Design review of the part built by this model. Coordinates are the model's own, in mm. A direction names the side the tool comes from. Give positions to 0.01 mm unless a question says otherwise; leave off trailing zeros. Loops run counter-clockwise (first coordinate to the right, second up) from the corner with the lowest first, then second, coordinate; pieces in that order, holes last. Notation, with made-up numbers: M 47.25,61 L 80.25,61 A19 ccw 80.25,81 Z; hole C -37.75,51.25 d3. An arc over 180 degrees is marked long. Use a Markdown table: item, result. Add a question column.
(1) Add section A-A, the plane x = -315. Give the boundary of the cut face in (y, z), then the cut area to 3 significant figures.
(2) Add section C-C, the plane y = -566. Give the boundary of the cut face in (x, z).
(3) Draft analysis for pull direction Y (two halves, no side actions). For faces 4 (the face through (0, -309, -7)), 5 (the face through (-358, 0, 38)), 6 (the face through (-355, -1, 75)), state which applies: pulls with the +Y half, pulls with the -Y half, needs draft (parallel to the pull), parting line crosses it, or undercut.
(4) Add section B-B, the plane x = -155. Give the boundary of the cut face in (y, z).
(5) Add section D-D, the plane y = -408.5. Give the boundary of the cut face in (x, z).
(6) For faces 1 (the face through (-348.058, -140.941, -14.953)), 2 (the face through (-707.014, -305.559, 5.517)), 3 (the face through (-358, -618, -33)), list the 3-axis set-ups (+Z, -Z, +X, -X, +Y, -Y) from which the entire face can be reached by the end or side of a thin tool; tool diameter is ignored.
(7) For probe 1 along X at (y, z) = (-585.5, -31); probe 2 along Y at (x, z) = (-285.5, 33.5); probe 3 along Z at (x, y) = (-283, -518), list the stretches that pass through material, from the lowest coordinate up.
(8) Insertion check: pin 1 Ø3 at (x, z) = (-502.5, 2.5) entering from +Y; pin 2 Ø1 at (x, y) = (1, -610.5) entering from +Z; pin 3 Ø10 at (x, y) = (-428.5, -477.5) entering from -Z. Each pin has a flat end and moves straight along its axis. Give the tip position at first contact, or say it passes through.
```python
from build123d import *

# Parameters (mm, degrees)
BOSS_EXTRUDE1_DEPTH = 2
BOSS_EXTRUDE2_DEPTH = 706
SKETCH3_W           = 706
SKETCH3_H           = 73
CUT_EXTRUDE1_DEPTH  = 940.955850027
BOSS_EXTRUDE3_START = 2
BOSS_EXTRUDE3_DEPTH = 2
CUT_EXTRUDE2_REACH  = 951.714
SKETCH5_W           = 628
SKETCH5_H           = 323
SKETCH6_W           = 100
SKETCH6_H           = 80
SKETCH6_W_2         = 344
CUT_EXTRUDE3_DEPTH  = 2
SKETCH7_W           = 706
SKETCH7_H           = 4
BOSS_EXTRUDE4_DEPTH = 61


with BuildPart() as part:
    # Sketch1 → Boss-Extrude1 (new body)
    with BuildSketch(Plane(origin=(0, 0, 0), x_dir=(0, 0, -1), z_dir=(1, 0, 0))):
        with BuildLine():
            Line((0, 0), (-75, 0))
            Line((-75, 0), (-75, -40))
            ThreePointArc((-75, -40), (-39.844354311, -53.471133381), (-31.447716035, -90.171096924))
            Line((-31.447716035, -90.171096924), (19.696734432, -515))
            Line((19.696734432, -515), (19.696734432, -543.691772505))
            ThreePointArc((19.696734432, -543.691772505), (13.304376378, -574.16353688), (-13, -590.820981133))
            Line((-13, -590.820981133), (-13, -618))
            Line((-13, -618), (62, -618))
            Line((62, -618), (62, -515))
            Line((62, -515), (0, 0))
        make_face()
    extrude(amount=BOSS_EXTRUDE1_DEPTH)

    # Sketch2 → Boss-Extrude2 (add)
    with BuildSketch(Plane.ZY):
        Polygon((13, -618), (-62, -618), (-62, -515), (0, 0), (75, 0), (75, -2), (1.773664518, -2), (-60, -515.119955274), (-60, -616), (13, -616), align=None)
    extrude(amount=BOSS_EXTRUDE2_DEPTH)

    # Sketch3 → Cut-Extrude1 (cut, through all)
    with BuildSketch(Plane(origin=(0, -616, 0), x_dir=(1, 0, 0), z_dir=(0, 1, 0))):
        with Locations((-353, 23.5)):
            Rectangle(SKETCH3_W, SKETCH3_H)
    extrude(amount=-CUT_EXTRUDE1_DEPTH, mode=Mode.SUBTRACT)

    # Sketch4 → Boss-Extrude3 (add)
    with BuildSketch(Plane.ZY.offset(706).offset(BOSS_EXTRUDE3_START)):
        with BuildLine():
            Line((-19.696734432, -543.691772505), (-19.696734432, -515))
            Line((-19.696734432, -515), (31.447716035, -90.171096924))
            ThreePointArc((31.447716035, -90.171096924), (39.844354311, -53.471133381), (75, -40))
            Line((75, -40), (75, 0))
            Line((75, 0), (0, 0))
            Line((0, 0), (-62, -515))
            Line((-62, -515), (-62, -618))
            Line((-62, -618), (13, -618))
            Line((13, -618), (13, -590.820981133))
            ThreePointArc((13, -590.820981133), (-13.304376378, -574.16353688), (-19.696734432, -543.691772505))
        make_face()
    extrude(amount=-BOSS_EXTRUDE3_DEPTH)

    # Cut-Extrude2: up to this plane
    cut_extrude2_end = Plane(origin=(-706, -515.119955274, -60), z_dir=(0, 0.1195253040577556, -0.9928311546732914))
    # Sketch5 → Cut-Extrude2 (cut, up to the surface)
    with BuildSketch(Plane(origin=(0, 0, -62), x_dir=(-1, 0, 0), z_dir=(0, 0, -1)), mode=Mode.PRIVATE) as cut_extrude2_sk1:
        with Locations((353, -313.5)):
            Rectangle(SKETCH5_W, SKETCH5_H)
    cut_extrude2_tool1 = split(extrude(cut_extrude2_sk1.sketch, amount=-CUT_EXTRUDE2_REACH, mode=Mode.PRIVATE), bisect_by=cut_extrude2_end, keep=Keep.BOTH, mode=Mode.PRIVATE)
    add(cut_extrude2_tool1.solids().sort_by_distance((-353, -313.5, -62))[0], mode=Mode.SUBTRACT)

    # Sketch6 → Cut-Extrude3 (cut)
    with BuildSketch(Plane(origin=(0, 0, -62), x_dir=(-1, 0, 0), z_dir=(0, 0, -1))):
        with Locations((97, -568)):
            Rectangle(SKETCH6_W, SKETCH6_H)
        with Locations((353, -568)):
            Rectangle(SKETCH6_W_2, SKETCH6_H)
    extrude(amount=-CUT_EXTRUDE3_DEPTH, mode=Mode.SUBTRACT)

    # Sketch7 → Boss-Extrude4 (add)
    with BuildSketch(Plane.XY.offset(-60)):
        with Locations((-353, -616)):
            Rectangle(SKETCH7_W, SKETCH7_H)
    extrude(amount=BOSS_EXTRUDE4_DEPTH)


solid = part.part
```
Established:
| question | item | result |
|---|---|---|
| 1 | outline | M -618,-62 L -608,-62 L -608,-60 L -614,-60 L -614,1 L -618,1 Z; M -528,-62 L -515,-62 L -475,-57.18 L -475,-55.17 L -515.12,-60 L -528,-60 Z; M -152,-18.3 L 0,0 L 0,75 L -2,75 L -2,1.77 L -152,-16.28 Z |
| 1 | area | 823 mm^2 |
| 2 | outline | M -708,-62 L -525,-62 L -525,-60 L -706,-60 L -706,-17.66 L -708,-17.66 Z; M -181,-62 L -147,-62 L -147,-60 L -181,-60 Z; M -47,-62 L 2,-62 L 2,-17.66 L 0,-17.66 L 0,-60 L -47,-60 Z |
| 3 | face 4 | undercut |
| 3 | face 5 | pulls with the +Y half |
| 3 | face 6 | needs draft |
| 4 | outline | M -618,-62 L -515,-62 L -475,-57.18 L -475,-55.17 L -515.12,-60 L -614,-60 L -614,1 L -618,1 Z; M -152,-18.3 L 0,0 L 0,75 L -2,75 L -2,1.77 L -152,-16.28 Z |
| 5 | outline | M -708,-49.18 L -667,-49.18 L -667,-47.16 L -706,-47.16 L -706,-6.88 L -708,-6.88 Z; M -39,-49.18 L 2,-49.18 L 2,-6.88 L 0,-6.88 L 0,-47.16 L -39,-47.16 Z |
| 6 | face 1 | +Z |
| 6 | face 2 | +Z, +X, -X |
| 6 | face 3 | +Z, -Z, +X, -X, -Y |
| 7 | probe 1 | -708 to -706, 0 to 2 |
| 7 | probe 2 | -2 to 0 |
| 7 | probe 3 | -62 to -60 |
| 8 | pin 1 | y = 0 |
| 8 | pin 2 | z = 13 |
| 8 | pin 3 | z = -58.09 |
